Input: part model. Units: mm. Frame: model coordinates. A direction names the side the tool comes from. Coordinates: 2 decimals unless noted, no trailing zeros. Write each loop counter-clockwise with the first axis right and the second up, starting at its lowest first coordinate (ties: lowest second). Pieces come first, ordered by that corner, then holes. Notation, with made-up numbers: (33, 45) - (49, 45) arc R19 ccw to (49, 79) - close; hole circle Ø2 at (78.5, 20.5). An arc over 180 degrees is marked (long way). Use a Markdown table: item, result. Add a question column.
Q1. Section query A-A (z = 0). Return the cut outline in (x, y).
Q2. Section query B-B (y = -1.5). Return the cut outline in (x, z).
Q3. Set-up query: faces 1 (the face through (44.42, 3.905, -0.867)), 2 (the face through (80, 0, 0)). Return all of +Z, -Z, +X, -X, +Y, -Y with unobstructed straight access to the full face (end or side cutting, diameter ignored); none if empty.
Q4. Material intervals for probe 1 along X at (y, z) = (0.75, -5); probe 2 along X at (y, z) = (-2.25, -2); probe 3 along Y at (x, z) = (37, 0), sorted ascending. Write a range as from..to.
Q5. Section query C-C (x = 59). Return the cut outline in (y, z), then the cut area to 3 significant figures.
Q6. Pin query (flat end, axial travel): P1, Ø2, axis at x = 28, z = 4.5, coming from the -Y side; P2, Ø3, axis at x = 37.5, y = 0, coming from the -Z side; P3, Ø4, axis at x = 12.5, y = 2.5, coming from the +Z side; P4, Ø6, axis at y = 2.5, z = 0, coming from the +X side. Return the tip coordinate at first contact, or that it passes through.
Q7. Section query D-D (z = -3.25). Return the cut outline in (x, y).
from build123d import *


with BuildPart() as part:
    # Stepped Shaft Profile → Stepped Shaft Revolve (revolve)
    with BuildSketch(Plane.XY, mode=Mode.PRIVATE) as stepped_shaft_revolve_sk:
        Polygon((0, 0), (0, 6), (14, 6), (14, 4), (74, 4), (74, 2.25), (80, 2.25), (80, 0), align=None)
    revolve(stepped_shaft_revolve_sk.sketch.rotate(Axis((0, 0, 0), (1, 0, 0)), 90), axis=Axis((0, 0, 0), (1, 0, 0)))


solid = part.part
Values follow:
| question | item | result |
|---|---|---|
| 1 | outline | (0, -6) - (14, -6) - (14, -4) - (74, -4) - (74, -2.25) - (80, -2.25) - (80, 2.25) - (74, 2.25) - (74, 4) - (14, 4) - (14, 6) - (0, 6) - close |
| 2 | outline | (0, -5.81) - (14, -5.81) - (14, -3.71) - (74, -3.71) - (74, -1.68) - (80, -1.68) - (80, 1.68) - (74, 1.68) - (74, 3.71) - (14, 3.71) - (14, 5.81) - (0, 5.81) - close |
| 3 | face 1 | +X |
| 3 | face 2 | +Z, -Z, +X, +Y, -Y |
| 4 | probe 1 | 0..14 |
| 4 | probe 2 | 0..74 |
| 4 | probe 3 | -4..4 |
| 5 | outline | circle Ø8 at (0, 0) |
| 5 | area | 50.3 mm2 |
| 6 | P1 | y = -1.94 |
| 6 | P2 | z = -4 |
| 6 | P3 | z = 5.98 |
| 6 | P4 | x = 80 |
| 7 | outline | (0, -5.04) - (14, -5.04) - (14, -2.33) - (74, -2.33) - (74, 2.33) - (14, 2.33) - (14, 5.04) - (0, 5.04) - close |
